The model under review builds one solid part; all positions refer to its coordinate system, in mm. A direction names the side the tool comes from. Round coordinates to 2 decimals unless told otherwise and drop trailing zeros. Order: outer loops, then holes, each group sorted by start corner. A loop starts at its lowest first (then second) coordinate and runs counter-clockwise, first axis right, second up. Notation, with made-up numbers: (36.5, 6) -> (79.5, 6) arc R24 cw to (79.5, 45) -> close; hole circle Ø9 at (22.5, 81.5). An arc over 180 degrees is marked (long way). Use a Markdown table: item, result. Add a question column.
```python
from build123d import *

# Parameters (mm, degrees)
BOSS_EXTRUDE1_DEPTH     = 20
CUT_EXTRUDE1_DEPTH      = 46
CUT_EXTRUDE1_DEPTH_BACK = 46
SKETCH2_R               = 4
SKETCH2_R_2             = 1
CUT_EXTRUDE3_DEPTH      = 46
CUT_EXTRUDE3_DEPTH_BACK = 46
SKETCH5_R               = 4
CUT_EXTRUDE4_DEPTH      = 38.749172176


with BuildPart() as part:
    # Sketch1 → Boss-Extrude1 (new body)
    with BuildSketch(Plane(origin=(0, 0, 0), x_dir=(1, 0, 0), z_dir=(0, 1, 0))):
        Polygon((0, 0), (25, 0), (25, 15), (35, 15), (35, 20), (0, 20), align=None)
    extrude(amount=BOSS_EXTRUDE1_DEPTH)

    # Sketch2 → Cut-Extrude1 (cut, two sides: drawn at the far end of the back side and taken through both)
    with BuildSketch(Plane.XY.offset(-CUT_EXTRUDE1_DEPTH_BACK)):
        with Locations((8.5, 10)):
            Circle(SKETCH2_R)
        with Locations((23, 10)):
            Circle(SKETCH2_R_2)
    extrude(amount=CUT_EXTRUDE1_DEPTH + CUT_EXTRUDE1_DEPTH_BACK, mode=Mode.SUBTRACT)

    # Sketch5 → Cut-Extrude3 (cut, two sides: drawn at the far end of the back side and taken through both)
    with BuildSketch(Plane(origin=(0, 20, 0), x_dir=(1, 0, 0), z_dir=(0, 1, 0)).offset(-CUT_EXTRUDE3_DEPTH_BACK)):
        with Locations(Location((8.5, 10, 0), (0, 0, 270))):
            Circle(SKETCH5_R)
    extrude(amount=CUT_EXTRUDE3_DEPTH + CUT_EXTRUDE3_DEPTH_BACK, mode=Mode.SUBTRACT)

    # Sketch6 → Cut-Extrude4 (cut, through all)
    with BuildSketch(Plane(origin=(25, 0, 0), x_dir=(0, 0, -1), z_dir=(1, 0, 0))):
        Polygon((2, 14), (2, 6), (8, 6), (8, 2.004568818), (15, 2.004568818), (15, 17.995431182), (8, 17.995431182), (8, 14), align=None)
    extrude(amount=-CUT_EXTRUDE4_DEPTH, mode=Mode.SUBTRACT)


solid = part.part
```
Q1. Wall thickness on line 1 (X direction, y = 10, z = -0.5); line 2 (X direction, y = 10, z = -16.25); line 3 (Y direction, x = 23, z = -17.85): over which ranges is each line inside the solid? List them lowest first. Write a range as [from, to].
Q2. Add section C-C (y = 10). Write out the cut boundary in (x, z).
Q3. Add section B-B (z = -14.5). Write out the cut boundary in (x, y).
Q4. Machinability: for faces 5 (the flat face through (35, 10, -17)), 6 (the flat face through (13, 14, -5)), which of the approach directions +Z, -Z, +X, -X, +Y, -Y give a long, thin tool a straight path to every point of the face, cutting with its end or side? Answer none if there is none.
Q5. Add section D-D (x = 23). Write out the cut boundary in (y, z).
Q6. Mouldability with a two-part tool opening along X and no side actions: class faces 1 (the flat face through (25, 5, -6)), 2 (the flat face through (0, 5, -6)), 3 (the flat face through (13, 17.995, -12)), 4 (the cylindrical face through (9.701, 2.291, -6.185)) as pulls with the +X half, pulls with the -X half, needs draft (parallel to the pull), parting line crosses it, or undercut.
Q7. Add section A-A (y = 17.25). Write out the cut boundary in (x, z), then the cut area to 3 significant figures.
Q8. Insertion check: pin 1 (3 mm diameter, centred on y = 16, z = -6, fed in from +X). The pin has a flat end and moves straight along its axis. Give the tip position at first contact, or say it passes through.
Report:
| question | item | result |
|---|---|---|
| 1 | line 1 | x = [0, 4.5], [12.5, 22], [24, 25] |
| 1 | line 2 | x = [0, 4.5], [12.5, 22], [24, 35] |
| 1 | line 3 | y = [0, 9], [11, 20] |
| 2 | outline | (0, -20) -> (4.5, -20) -> (4.5, -15) -> (0, -15) -> close; (0, -2) -> (4.5, -2) -> (4.5, 0) -> (0, 0) -> close; (12.5, -20) -> (22, -20) -> (22, -15) -> (12.5, -15) -> close; (12.5, -2) -> (22, -2) -> (22, 0) -> (12.5, 0) -> close; (24, -20) -> (35, -20) -> (35, -15) -> (24, -15) -> close; (24, -2) -> (25, -2) -> (25, 0) -> (24, 0) -> close |
| 3 | outline | (0, 0) -> (25, 0) -> (25, 2) -> (0, 2) -> close; (0, 18) -> (25, 18) -> (25, 20) -> (0, 20) -> close |
| 4 | face 5 | +Z, -Z, +X, +Y, -Y |
| 4 | face 6 | +X, -X |
| 5 | outline | (0, -20) -> (9, -20) -> (9, -15) -> (2, -15) -> (2, -8) -> (6, -8) -> (6, -2) -> (9, -2) -> (9, 0) -> (0, 0) -> close; (11, -20) -> (20, -20) -> (20, 0) -> (11, 0) -> (11, -2) -> (14, -2) -> (14, -8) -> (18, -8) -> (18, -15) -> (11, -15) -> close |
| 6 | face 1 | pulls with the +X half |
| 6 | face 2 | pulls with the -X half |
| 6 | face 3 | needs draft |
| 6 | face 4 | undercut |
| 7 | outline | (0, -20) -> (35, -20) -> (35, -15) -> (0, -15) -> close; (0, -8) -> (5.04, -8) arc R4 cw to (11.96, -8) -> (25, -8) -> (25, 0) -> (0, 0) -> close |
| 7 | area | 365 mm² |
| 8 | pin 1 | stops at x = 25 |
